Part print with two shaded views. Sizes in mm from the minimum x, y, z corner. Round coordinates to 2 decimals unless told otherwise and drop trailing zeros. Loops run counter-clockwise (first coordinate to the right, second up) from the corner with the lowest first, then second, coordinate; pieces in that order, holes last. Notation, with made-up numbers: (84, 76) - (88, 76) arc R29 cw to (88, 111) - close; hole circle Ø4 at (-10, 72.5). An arc over 180 degrees is marked (long way). Write each question's results on one line, items separated by ' | '. Start each with the question number.
(1) Flat gauge pins, fed straight in: P1, Ø2, axis at x = 13, y = 13, coming from the -Z side; P2, Ø1, axis at x = 6, y = 9, coming from the +Z side; P3, Ø2, axis at x = 14, z = 2, coming from the +Y side; P4, Ø1.5, axis at x = 12, z = 2.5, coming from the +Y side. Where does each tip first touch, or does it go through?
(2) Mould opens along Y. For the marked faces 1, 2 and 3 say: released by +Y, released by -Y, zero draft, split by the parting line, or undercut.
(3) Cut at B-B, the plane z = 1.3. List the corners of the cut face in (x, y).
(4) Cut at A-A, the plane x = 10.75. List the corners of the cut face in (y, z).
(5) Drill centre lines: L1, parallel to Y at x = 10.75, z = 1.9; L2, parallel to X at y = 10.5, z = 2.55; L3, parallel to X at y = 12.25, z = 1.15. Where is each one in solid material? Low to high.
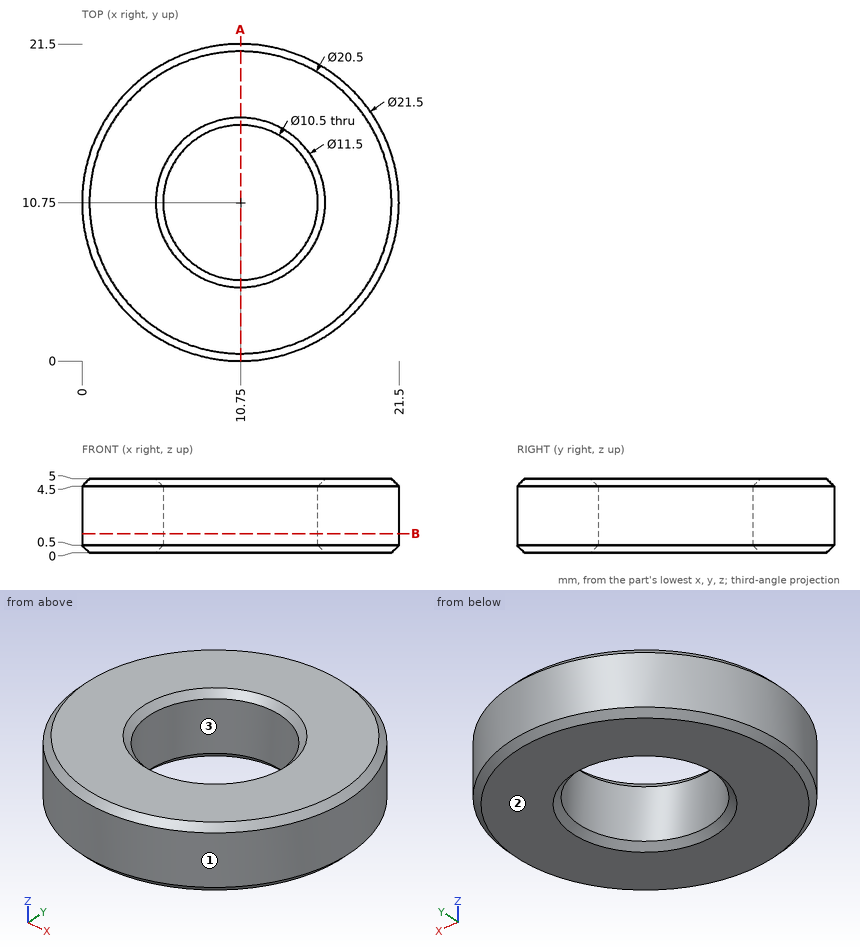
A:
1) P1: through | P2: z = 4.81 | P3: y = 21.26 | P4: y = 21.49
2) face 1: split by the parting line | face 2: zero draft | face 3: undercut
3) outline: circle Ø21.5 at (10.75, 10.75); hole circle Ø10.5 at (10.75, 10.75)
4) outline: (0, 0.5) - (0.5, 0) - (5, 0) - (5.5, 0.5) - (5.5, 4.5) - (5, 5) - (0.5, 5) - (0, 4.5) - close; (16, 0.5) - (16.5, 0) - (21, 0) - (21.5, 0.5) - (21.5, 4.5) - (21, 5) - (16.5, 5) - (16, 4.5) - close
5) L1: 0 to 5.5, 16 to 21.5 | L2: 0 to 5.51, 15.99 to 21.5 | L3: 0.11 to 5.72, 15.78 to 21.39
